from build123d import *

# Parameters (mm, degrees)
SKETCH1_R           = 8
BOSS_EXTRUDE1_DEPTH = 8


with BuildPart() as part:
    # Sketch1 → Boss-Extrude1 (new body)
    with BuildSketch(Plane.XY):
        with BuildLine():
            Line((0, 0), (0, 40))
            Line((0, 40), (27.338105329, 83.042165339))
            ThreePointArc((27.338105329, 83.042165339), (40, 90), (52.661894671, 83.042165339))
            Line((52.661894671, 83.042165339), (80, 40))
            Line((80, 40), (80, 0))
            Line((80, 0), (0, 0))
        make_face()
        with Locations((40, 75)):
            Circle(SKETCH1_R, mode=Mode.SUBTRACT)
    extrude(amount=BOSS_EXTRUDE1_DEPTH)


solid = part.part
Work out the finished part from the listing and answer in its coordinate system (mm). Give positions to 0.01 mm unless a question says otherwise; leave off trailing zeros. Write each loop counter-clockwise with the first axis right and the second up, starting at its lowest first coordinate (ties: lowest second). Pieces come first, ordered by that corner, then holes. Notation, with made-up numbers: (38, 83.5) - (89, 83.5) arc R10 ccw to (89, 90.5) - close; hole circle Ø1 at (-23, -13.75). An arc over 180 degrees is marked (long way). One line per item, written item: value. Start each with the question number.
1. Find section A-A (x = 40). Write down the section's boundary in (y, z).
2. Find section B-B (z = 5.5). Write down the section's boundary in (x, y), then the cut area to 3 significant figures.
3. Consider probe 1 along Y at (x, z) = (40, 4); probe 2 along Y at (x, z) = (46.5, 4.75); probe 3 along Y at (x, z) = (66, 6.25). Determine where each line is inside the solid, lowest interval first.
4. Given pin 1 (1 mm diameter, centred on x = 66, z = 6, fed in from +Y); pin 2 (9.5 mm diameter, centred on x = 40, y = 75, fed in from -Z); pin 3 (2 mm diameter, centred on y = 64.5, z = 6.5, fed in from -X), each flat-ended and moving along its own axis, determine where each tip first touches the part or whether it passes through.
5. For a pull along Y with two mould halves and no side action, classify faces 1 (the cylindrical face through (40, 90, 4)), 2 (the cylindrical face through (38.959, 82.932, 3.944)), 3 (the flat face through (41, 36, 8)) as +Y half, -Y half, draft (parallel to the pull), parting line (faces both ways), or undercut.
6. Find section D-D (y = 59). Write down the section's boundary in (x, z).
7. Find section C-C (y = 81). Write down the section's boundary in (x, z).
Geometry results:
1. outline: (0, 0) - (67, 0) - (67, 8) - (0, 8) - close; (83, 0) - (90, 0) - (90, 8) - (83, 8) - close
2. outline: (0, 0) - (80, 0) - (80, 40) - (52.66, 83.04) arc R15 ccw to (27.34, 83.04) - (0, 40) - close; hole circle Ø16 at (40, 75)
2. area: 5,390 mm2
3. probe 1: 0 to 67, 83 to 90
3. probe 2: 0 to 70.34, 79.66 to 88.52
3. probe 3: 0 to 62.04
4. pin 1: y = 62.83
4. pin 2: through
4. pin 3: x = 14.93
5. face 1: +Y half
5. face 2: undercut
5. face 3: draft
6. outline: (12.07, 0) - (67.93, 0) - (67.93, 8) - (12.07, 8) - close
7. outline: (26.04, 0) - (34.71, 0) - (34.71, 8) - (26.04, 8) - close; (45.29, 0) - (53.96, 0) - (53.96, 8) - (45.29, 8) - close
